The model under review builds one solid part; all positions refer to its coordinate system, in mm. Coordinates: 2 decimals unless noted, no trailing zeros. Use one line per item in the form item = value. Start each with the question number.
```python
from build123d import *

# Parameters (mm, degrees)
SKETCH_1_R      = 2.1
SKETCH_1_R_2    = 3.4
EXTRUDE_1_DEPTH = 620


with BuildPart() as part:
    # 草图1 → 拉伸1 (new body)
    with BuildSketch(Plane(origin=(0, 0, 0), x_dir=(1, 0, 0), z_dir=(0, 1, 0))):
        with BuildLine():
            Line((6.75, -28), (11, -28))
            Line((11, -28), (11, -30))
            Line((11, -30), (2, -30))
            ThreePointArc((2, -30), (0.585786438, -29.414213562), (0, -28))
            Line((0, -28), (0, -19))
            Line((0, -19), (2, -19))
            Line((2, -19), (2, -23.25))
            Line((2, -23.25), (5.335785999, -23.25))
            Line((5.335785999, -23.25), (9, -19.585785999))
            Line((9, -19.585785999), (9, -10.414214001))
            Line((9, -10.414214001), (5.335785999, -6.75))
            Line((5.335785999, -6.75), (2, -6.75))
            Line((2, -6.75), (2, -11))
            Line((2, -11), (0, -11))
            Line((0, -11), (0, -2))
            ThreePointArc((0, -2), (0.585786438, -0.585786438), (2, 0))
            Line((2, 0), (11, 0))
            Line((11, 0), (11, -2))
            Line((11, -2), (6.75, -2))
            Line((6.75, -2), (6.75, -5.335785999))
            Line((6.75, -5.335785999), (10.414214001, -9))
            Line((10.414214001, -9), (19.585785999, -9))
            Line((19.585785999, -9), (23.25, -5.335785999))
            Line((23.25, -5.335785999), (23.25, -2))
            Line((23.25, -2), (19, -2))
            Line((19, -2), (19, 0))
            Line((19, 0), (28, 0))
            ThreePointArc((28, 0), (29.414213562, -0.585786438), (30, -2))
            Line((30, -2), (30, -11))
            Line((30, -11), (28, -11))
            Line((28, -11), (28, -6.75))
            Line((28, -6.75), (24.664214001, -6.75))
            Line((24.664214001, -6.75), (21, -10.414214001))
            Line((21, -10.414214001), (21, -19.585785999))
            Line((21, -19.585785999), (24.664214001, -23.25))
            Line((24.664214001, -23.25), (28, -23.25))
            Line((28, -23.25), (28, -19))
            Line((28, -19), (30, -19))
            Line((30, -19), (30, -28))
            ThreePointArc((30, -28), (29.414213562, -29.414213562), (28, -30))
            Line((28, -30), (19, -30))
            Line((19, -30), (19, -28))
            Line((19, -28), (23.25, -28))
            Line((23.25, -28), (23.25, -24.664214001))
            Line((23.25, -24.664214001), (19.585785999, -21))
            Line((19.585785999, -21), (10.414214001, -21))
            Line((10.414214001, -21), (6.75, -24.664214001))
            Line((6.75, -24.664214001), (6.75, -28))
        make_face()
        with Locations(Location((3.375, -26.625, 0), (0, 0, 270))):
            Circle(SKETCH_1_R, mode=Mode.SUBTRACT)
        with Locations(Location((26.625, -26.625, 0), (0, 0, 270))):
            Circle(SKETCH_1_R, mode=Mode.SUBTRACT)
        with Locations(Location((15, -15, 0), (0, 0, 270))):
            Circle(SKETCH_1_R_2, mode=Mode.SUBTRACT)
        with Locations(Location((3.375, -3.375, 0), (0, 0, 270))):
            Circle(SKETCH_1_R, mode=Mode.SUBTRACT)
        with Locations(Location((26.625, -3.375, 0), (0, 0, 270))):
            Circle(SKETCH_1_R, mode=Mode.SUBTRACT)
    extrude(amount=EXTRUDE_1_DEPTH)


solid = part.part
```
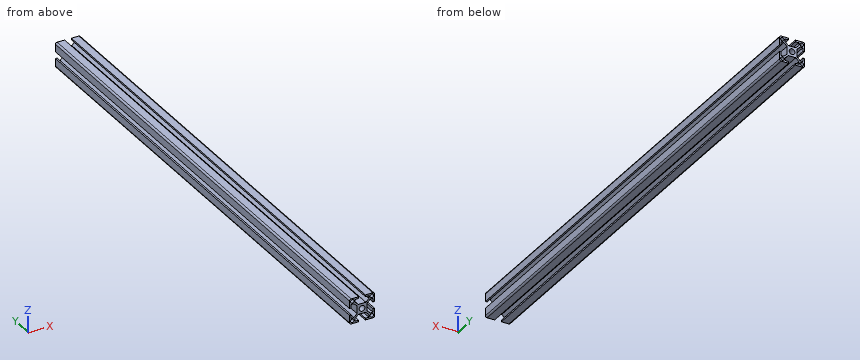
1. For P1, Ø1.6, axis at y = 341, z = 1, coming from the -X side; P2, Ø1, axis at y = 236.5, z = 29, coming from the +X side; P3, Ø0.6, axis at x = 28.5, y = 205.5, coming from the +Z side, all flat-tipped, find the tip position at first contact; note any pin that passes through.
2. For L1, parallel to Z at x = 27, y = 566; L2, parallel to X at y = 294, z = 14.5; L3, parallel to X at y = 312, z = 3.5, list the stretches that pass through material, from the lowest coordinate up.
3. Take a section at A-A (y = 150). Count the separate pieces of the cut face and the enclosed holes in it, plus the area to 3 significant figures.
Returned:
q1.P1 = 0.01
q1.P2 = 29.94
q1.P3 = 29.99
q2.L1 = 0 to 1.31, 5.44 to 6.75, 23.25 to 24.56, 28.69 to 30
q2.L2 = 9 to 11.64, 18.36 to 21
q2.L3 = 0 to 1.28, 5.47 to 6.75, 23.25 to 24.53, 28.72 to 30
q3.separate_pieces = 1
q3.enclosed_holes = 5
q3.area = 333 mm²
